from build123d import *

# Parameters (mm, degrees)
SKETCH1_W              = 120
SKETCH1_H              = 80
BOSS_EXTRUDE1_DEPTH    = 25
M12_TAPPED_HOLE1_D     = 10.2
M12_TAPPED_HOLE1_DEPTH = 29.25
M12_TAPPED_HOLE1_TIP   = 3.064389157


with BuildPart() as part:
    # Sketch1 → Boss-Extrude1 (new body)
    with BuildSketch(Plane.XY):
        Rectangle(SKETCH1_W, SKETCH1_H)
    extrude(amount=BOSS_EXTRUDE1_DEPTH)

    # M12 Tapped Hole1
    with Locations(Plane.XY.offset(25)):
        with Locations((-35, 7), (35, 7)):
            Hole(M12_TAPPED_HOLE1_D / 2, depth=M12_TAPPED_HOLE1_DEPTH)
            with Locations((0, 0, -(M12_TAPPED_HOLE1_DEPTH + M12_TAPPED_HOLE1_TIP / 2))):  # 118° drill point
                Cone(0, M12_TAPPED_HOLE1_D / 2, M12_TAPPED_HOLE1_TIP, mode=Mode.SUBTRACT)


solid = part.part
Input: part model. Units: mm. Frame: model coordinates. Coordinates: 2 decimals unless noted, no trailing zeros. Loops run counter-clockwise (first coordinate to the right, second up) from the corner with the lowest first, then second, coordinate; pieces in that order, holes last.
(1) Material intervals for probe 1 along Y at (x, z) = (35, 15.75); probe 2 along X at (y, z) = (10, 11.5); probe 3 along Y at (x, z) = (-32, 20.5), sorted ascending.
(2) Section C-C on z = 11.75. Return the cut outline in (x, y).
(3) First-contact query: pin 1 Ø6 at (x, y) = (-35, 7) entering from -Z. Flat tip, straight axial feed; report the tip coordinate or a pass-through.
(4) Section A-A on x = 35. Return the cut outline in (y, z), then the cut area to 4 significant figures.
(5) Pull-direction query (X, two-part tool) for faces 1 (the face through (-60, -1, 12)), 2 (the face through (60, -1, 12)), 3 (the face through (38.8, 10.4, 12.3)), 4 (the face through (-1, 1, 25)); classes: released by +X, released by -X, zero draft, split by the parting line, or undercut.
(6) Section B-B on y = 7. Return the cut outline in (x, z), then the cut area to 3 significant figures.
Data:
1. probe 1: y = -40 to 1.9, 12.1 to 40
1. probe 2: x = -60 to -39.12, -30.88 to 30.88, 39.12 to 60
1. probe 3: y = -40 to 2.88, 11.12 to 40
2. outline: (-60, -40) - (60, -40) - (60, 40) - (-60, 40) - close; hole circle Ø10.2 at (-35, 7); hole circle Ø10.2 at (35, 7)
3. pin 1: passes through
4. outline: (-40, 0) - (1.9, 0) - (1.9, 25) - (-40, 25) - close; (12.1, 0) - (40, 0) - (40, 25) - (12.1, 25) - close
4. area: 1,745 mm2
5. face 1: released by -X
5. face 2: released by +X
5. face 3: undercut
5. face 4: zero draft
6. outline: (-60, 0) - (-40.1, 0) - (-40.1, 25) - (-60, 25) - close; (-29.9, 0) - (29.9, 0) - (29.9, 25) - (-29.9, 25) - close; (40.1, 0) - (60, 0) - (60, 25) - (40.1, 25) - close
6. area: 2,490 mm2
